The listing builds one solid part. Answer for the finished solid, in the listing's coordinates (mm). Face numbers are marked on the shaded views. A direction names the side the tool comes from. Round coordinates to 2 decimals unless told otherwise and drop trailing zeros. Write each loop counter-clockwise with the first axis right and the second up, starting at its lowest first coordinate (ties: lowest second). Pieces come first, ordered by that corner, then holes. Notation, with made-up numbers: M -18.5,83 L 40.5,83 A17 ccw 40.5,100 Z; hole C -37.75,-14 d9. An arc over 180 degrees is marked long. Put each result on its own line as item: value. Start each with the question number.
```python
from build123d import *

# Parameters (mm, degrees)
BOSS_EXTRUDE1_DEPTH    = 50
CHAMFER2_SIZE          = 2
HOLE4_D                = 9
HOLE4_CBORE_D          = 15
HOLE4_CBORE_DEPTH      = 10
M14X1_5_TAPPED_HOLE1_D = 12.5
M12_TAPPED_HOLE1_D     = 10.2


with BuildPart() as part:
    # Sketch1 → Boss-Extrude1 (new body)
    with BuildSketch(Plane.XY):
        Polygon((-40.819758101, 19.90625), (-40.819758101, -27.59375), (-0.819758101, -27.59375), (-0.819758101, -12.59375), (-25.819758101, -12.59375), (-25.819758101, 19.90625), align=None)
    extrude(amount=BOSS_EXTRUDE1_DEPTH)

    # Chamfer2
    chamfer2_edges = [part.edges().sort_by_distance(p)[0] for p in [
        (-0.819758101, -20.09375, 50),
        (-33.319758101, 19.90625, 50),
        (-0.819758101, -20.09375, 0),
        (-33.319758101, 19.90625, 0),
    ]]
    chamfer(chamfer2_edges, length=CHAMFER2_SIZE)

    # Hole4 (through all)
    with Locations(Plane(origin=(0, -12.59375, 0), x_dir=(1, 0, 0), z_dir=(0, 1, 0))):
        with Locations((-11.819758101, -10), (-11.819758101, -40)):
            CounterBoreHole(HOLE4_D / 2, HOLE4_CBORE_D / 2, HOLE4_CBORE_DEPTH)

    # M14x1.5 Tapped Hole1 (through all)
    with Locations(Plane(origin=(-25.819758101, 0, 0), x_dir=(0, 0, -1), z_dir=(1, 0, 0))):
        with Locations((-40, 6.90625)):
            Hole(M14X1_5_TAPPED_HOLE1_D / 2)

    # M12 Tapped Hole1 (through all)
    with Locations(Plane(origin=(-25.819758101, 0, 0), x_dir=(0, 0, -1), z_dir=(1, 0, 0))):
        with Locations((-9, 7.90625)):
            Hole(M12_TAPPED_HOLE1_D / 2)


solid = part.part
```
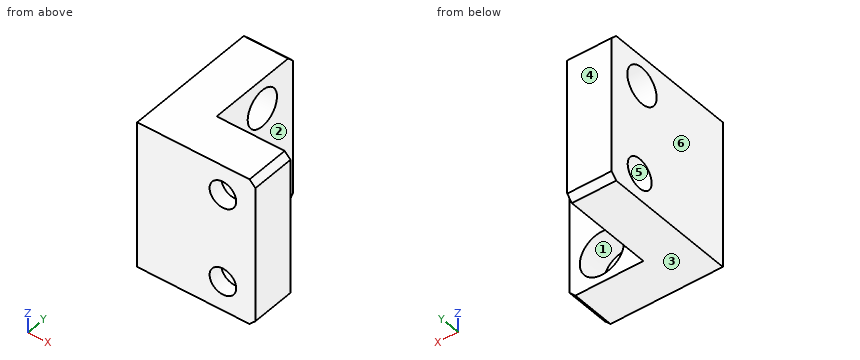
Item 1: Section C-C (z = 16) is taken. Give the vertices of the cut face in (x, y), and give its area (4 significant figures).
Item 2: Flat-ended cylindrical pins translate along their axes: pin 1 (7.5 mm diameter, centred on y = 6.91, z = 40, fed in from +X); pin 2 (16.5 mm diameter, centred on x = -13, z = 37, fed in from +Y); pin 3 (10.5 mm diameter, centred on x = -11.82, z = 40, fed in from +Y); pin 4 (16 mm diameter, centred on y = 9.5, z = 33, fed in from +X). Find the tip coordinate at first contact, or state that the pin passes through.
Item 3: Which of the six approach directions +Z, -Z, +X, -X, +Y, -Y give full straight-line access (tool end or side, diameter ignored) to the marked faces 1, 2 and 3?
Item 4: Section B-B (y = -24) is taken. Give the vertices of the cut face in (x, z), and give its area (3 significant figures).
Item 5: Determine the mould class of the marked faces 4, 5 and 6 for opening direction Y: released by +Y, released by -Y, zero draft, split by the parting line, or undercut.
Item 6: Section A-A (z = 40) is taken. Give the vertices of the cut face in (x, y), and give its area (3 significant figures).
Item 7: Section D-D (x = -29) is taken. Give the vertices of the cut face in (y, z), and give its area (3 significant figures).
Item 8: Consider line 1 along Y through (x, z) = (-29, 9); line 2 along Y through (x, z) = (-20, 10.5); line 3 along X through (y, z) = (-4.5, 39). Determine where each line is inside the solid, lowest interval first. Write a range as [from, to].
Output values:
1. outline: M -40.82,-27.59 L -0.82,-27.59 L -0.82,-12.59 L -7.32,-12.59 L -7.32,-22.59 L -16.32,-22.59 L -16.32,-12.59 L -25.82,-12.59 L -25.82,19.91 L -40.82,19.91 Z
1. area: 997.5 mm^2
2. pin 1: passes through
2. pin 2: stops at y = -12.59
2. pin 3: stops at y = -22.59
2. pin 4: stops at x = -25.82
3. face 1: +Y
3. face 2: +Z, -Z, +X, +Y
3. face 3: -Z, +X, -X, +Y, -Y
4. outline: M -40.82,0 L -2.82,0 L -0.82,2 L -0.82,48 L -2.82,50 L -40.82,50 Z; hole C -11.82,10 d9; hole C -11.82,40 d9
4. area: 1,870 mm^2
5. face 4: released by +Y
5. face 5: undercut
5. face 6: zero draft
6. outline: M -40.82,-27.59 L -16.32,-27.59 L -16.32,-22.59 L -19.32,-22.59 L -19.32,-12.59 L -25.82,-12.59 L -25.82,0.66 L -40.82,0.66 Z; M -40.82,13.16 L -25.82,13.16 L -25.82,19.91 L -40.82,19.91 Z; M -7.32,-27.59 L -0.82,-27.59 L -0.82,-12.59 L -4.32,-12.59 L -4.32,-22.59 L -7.32,-22.59 Z
6. area: 705 mm^2
7. outline: M -27.59,0 L 17.91,0 L 19.91,2 L 19.91,48 L 17.91,50 L -27.59,50 Z; hole C 6.91,40 d12.5; hole C 7.91,9 d10.2
7. area: 2,170 mm^2
8. line 1: y = [-27.59, 2.81], [13.01, 19.91]
8. line 2: y = [-27.59, -12.59]
8. line 3: x = [-40.82, -25.82]
